from build123d import *

# Parameters (mm, degrees)
V_BLOCK_BASE_DEPTH         = 70
V_BLOCK_BASE_DEPTH_BACK    = 30
CLAMP_ARCH_DEPTH           = 10
CLAMP_ARCH_FILLET_R2_R     = 2
CLAMP_SCREW_SKETCH_R       = 6
CLAMP_SCREW_SHAFT_DEPTH    = 60
CLAMP_START                = 40
SKETCH4_3_R                = 12
SKETCH4_3_R_2              = 6
CLAMP_SCREW_KNOB_DEPTH     = 20
KNOB_CROSS_HOLE_DEPTH      = 157.384142419
KNOB_CROSS_HOLE_DEPTH_BACK = 157.384142419
KNOB_CROSS_HOLE_SKETCH_R   = 2.5


with BuildPart() as part:
    # V-Block Profile Sketch → V-Block Base (new, two sides: drawn at the far end of the back side and taken through both)
    with BuildSketch(Plane.XY.offset(-V_BLOCK_BASE_DEPTH_BACK)):
        Polygon((-24, -6), (-30, -6), (-30, -30), (-20, -30), (-3.218007376, -10), (3.218007376, -10), (20, -30), (30, -30), (30, -6), (24, -6), (24, 6), (30, 6), (30, 30), (20, 30), (3.218007376, 10), (-3.218007376, 10), (-20, 30), (-30, 30), (-30, 6), (-24, 6), align=None)
    extrude(amount=V_BLOCK_BASE_DEPTH + V_BLOCK_BASE_DEPTH_BACK)

    # Clamp Arch Sketch → Clamp Arch (add, symmetric)
    with BuildSketch(Plane.XY):
        with BuildLine():
            Line((-40, -6), (40, -6))
            Line((40, -6), (40, 30))
            Line((40, 30), (36, 30))
            ThreePointArc((36, 30), (29.393876913, 50.784609691), (12, 63.941125497))
            Line((12, 63.941125497), (12, 74))
            Line((12, 74), (-12, 74))
            Line((-12, 74), (-12, 63.941125497))
            ThreePointArc((-12, 63.941125497), (-29.393876913, 50.784609691), (-36, 30))
            Line((-36, 30), (-40, 30))
            Line((-40, 30), (-40, -6))
        make_face()
        with BuildLine():
            Line((-20, 30), (-24, 30))
            ThreePointArc((-24, 30), (0, 54), (24, 30))
            Line((24, 30), (20, 30))
            Line((20, 30), (3.218007376, 10))
            Line((3.218007376, 10), (-3.218007376, 10))
            Line((-3.218007376, 10), (-20, 30))
        make_face(mode=Mode.SUBTRACT)
    extrude(amount=CLAMP_ARCH_DEPTH, both=True)

    # Clamp Arch Fillet R2
    clamp_arch_fillet_r2_edges = [part.edges().sort_by_distance(p)[0] for p in [
        (36, 30, 0),
        (12, 63.941125497, 0),
        (-12, 63.941125497, 0),
        (-36, 30, 0),
    ]]
    fillet(clamp_arch_fillet_r2_edges, radius=CLAMP_ARCH_FILLET_R2_R)

    # Clamp Screw Sketch → Clamp Screw Shaft (add)
    with BuildSketch(Plane(origin=(0, 74, 0), x_dir=(1, 0, 0), z_dir=(0, 1, 0))):
        with Locations(Location((0, 0, 0), (0, 0, 270))):
            Circle(CLAMP_SCREW_SKETCH_R)
    extrude(amount=CLAMP_SCREW_SHAFT_DEPTH)

    # Sketch4_3 → Clamp Screw Knob (add)
    with BuildSketch(Plane(origin=(0, 74, 0), x_dir=(1, 0, 0), z_dir=(0, 1, 0)).offset(CLAMP_START)):
        with Locations(Location((0, 0, 0), (0, 0, 270))):
            Circle(SKETCH4_3_R)
        with Locations(Location((0, 0, 0), (0, 0, 270))):
            Circle(SKETCH4_3_R_2, mode=Mode.SUBTRACT)
    extrude(amount=CLAMP_SCREW_KNOB_DEPTH)

    # Knob Cross Hole Sketch → Knob Cross Hole (cut, two sides: drawn at the far end of the back side and taken through both)
    with BuildSketch(Plane(origin=(0, 0, 0), x_dir=(0, 0, -1), z_dir=(1, 0, 0)).offset(-KNOB_CROSS_HOLE_DEPTH_BACK)):
        with Locations((0, 124)):
            Circle(KNOB_CROSS_HOLE_SKETCH_R)
    extrude(amount=KNOB_CROSS_HOLE_DEPTH + KNOB_CROSS_HOLE_DEPTH_BACK, mode=Mode.SUBTRACT)


solid = part.part
Geometry: final body of the model. Coordinates: model frame, mm. A direction names the side the tool comes from. Coordinates: 2 decimals unless noted, no trailing zeros. Order: outer loops, then holes, each group sorted by start corner. A loop starts at its lowest first (then second) coordinate and runs counter-clockwise, first axis right, second up. Notation, with made-up numbers: M -36,5.5 L 13,5.5 A24 cw 13,21.5 Z; hole C 22,68 d1. An arc over 180 degrees is marked long. One line per question, with ' | ' between items. Start each with the question number.
Item 1: Ray query, probe 1 along Y at (x, z) = (5, 0); probe 2 along Z at (x, y) = (-32.5, 33.5); probe 3 along Y at (x, z) = (-26, -18). Return the intervals inside material, ascending. Write a range as [from, to].
Item 2: Cut plane C-C, the plane z = 27.5. Return the cut outline in (x, y).
Item 3: Set-up query: faces 3 (the flat face through (0, 74, 7)), 4 (the flat face through (-11.49, 19.86, 19.3)), 5 (the flat face through (-24, 0, 40)), 6 (the flat face through (11.49, -19.86, 19.3)), 7 (the flat face through (30, -18, 19)). Return all of +Z, -Z, +X, -X, +Y, -Y with unobstructed straight access to the full face (end or side cutting, diameter ignored); none if empty.
Item 4: Cut plane B-B, the plane x = 15. Return the cut outline in (y, z) (3 decimals).
Item 5: Cut plane D-D, the plane y = -4. Return the cut outline in (x, z).
Item 6: Draft query along Z for faces 1 (the flat face through (-30, 18, 40)), 2 (the cylindrical face through (-0.17, 126.48, 0.33)). Return one class per face: released by +Z, released by -Z, zero draft, split by the parting line, or undercut.
Item 7: Pin query (flat end, axial travel): pin 1 Ø12 at (y, z) = (-12.5, 18.5) entering from -X; pin 2 Ø3 at (x, z) = (-0.5, 17) entering from -Y; pin 3 Ø6 at (y, z) = (-0.5, 49) entering from -X; pin 4 Ø24 at (x, y) = (0, 26) entering from +Z. Return the tip coordinate at first contact, or that it passes through.
Item 8: Cut plane A-A, the plane x = 0. Return the cut outline in (y, z), then the cut area to 3 significant figures.
A:
1) probe 1: y = [-12.12, 12.12], [53.47, 121.5], [126.5, 134] | probe 2: z = [-10, 10] | probe 3: y = [-30, -6], [6, 30]
2) outline: M -30,-30 L -20,-30 L -3.22,-10 L 3.22,-10 L 20,-30 L 30,-30 L 30,-6 L 24,-6 L 24,6 L 30,6 L 30,30 L 20,30 L 3.22,10 L -3.22,10 L -20,30 L -30,30 L -30,6 L -24,6 L -24,-6 L -30,-6 Z
3) face 3: none | face 4: +Z, -Z | face 5: +Z, -X | face 6: +Z, -Z, -Y | face 7: +Z, -Z, +X, -Y
4) outline: M -24.041,-30 L 24.041,-30 L 24.041,70 L -24.041,70 Z; M 48.735,-10 L 62.726,-10 L 62.726,10 L 48.735,10 Z
5) outline: M -40,-10 L -24,-10 L -24,-30 L 24,-30 L 24,-10 L 40,-10 L 40,10 L 24,10 L 24,70 L -24,70 L -24,10 L -40,10 Z
6) face 1: zero draft | face 2: undercut
7) pin 1: stops at x = -30 | pin 2: stops at y = -10 | pin 3: stops at x = -24 | pin 4: passes through
8) outline: M -10,-30 L 10,-30 L 10,70 L -10,70 Z; M 54,-10 L 74,-10 L 74,-6 L 114,-6 L 114,-12 L 134,-12 L 134,12 L 114,12 L 114,6 L 74,6 L 74,10 L 54,10 Z; hole C 124,0 d5 | area: 3,340 mm2
